```python
from build123d import *

# Parameters (mm, degrees)
BOSS_EXTRUDE1_DEPTH = 3.2
SKETCH8_R           = 2
CUT_EXTRUDE1_DEPTH  = 7.23083729


with BuildPart() as part:
    # Sketch1 → Boss-Extrude1 (new body)
    with BuildSketch(Plane(origin=(0, 0, 0), x_dir=(1, 0, 0), z_dir=(0, 1, 0))):
        Polygon((0, 4.041451884), (-3.5, 2.020725942), (-3.5, -2.020725942), (0, -4.041451884), (3.5, -2.020725942), (3.5, 2.020725942), align=None)
    extrude(amount=BOSS_EXTRUDE1_DEPTH)

    # Sketch3 → Cut-Revolve2 (revolve, cut)
    with BuildSketch(Plane(origin=(0, 0, 0), x_dir=(0.8660254037844417, 0, 0.4999999999999949), z_dir=(-0.4999999999999949, 0, 0.8660254037844417)), mode=Mode.PRIVATE) as cut_revolve2_sk:
        Polygon((4.041451884, 3.2), (4.041451884, 2.54), (3.381451884, 3.2), align=None)
        Polygon((4.041451884, 0), (4.041451884, 0.66), (3.381451884, 0), align=None)
    revolve(cut_revolve2_sk.sketch.rotate(Axis((0, -1.01584762, 0), (0, 1, 0)), 300), axis=Axis((0, -1.01584762, 0), (0, 1, 0)), mode=Mode.SUBTRACT)

    # Sketch8 → Cut-Extrude1 (cut, through all)
    with BuildSketch(Plane(origin=(0, 3.2, 0), x_dir=(1, 0, 0), z_dir=(0, 1, 0))):
        with Locations(Location((0, 0, 0), (0, 0, 270))):
            Circle(SKETCH8_R)
    extrude(amount=-CUT_EXTRUDE1_DEPTH, mode=Mode.SUBTRACT)


solid = part.part
```
The model under review builds one solid part; all positions refer to its coordinate system, in mm. Round coordinates to 2 decimals unless told otherwise and drop trailing zeros. Order: outer loops, then holes, each group sorted by start corner. A loop starts at its lowest first (then second) coordinate and runs counter-clockwise, first axis right, second up. Notation, with made-up numbers: (87.5, 51.5) -> (99.5, 51.5) arc R13 ccw to (99.5, 56.5) -> close; hole circle Ø5 at (70.25, 79). An arc over 180 degrees is marked (long way). One line per item, written item: value. Start each with the question number.
Q1. Clearance check with flat-ended pins moving along their axes: pin 1 Ø1 at (x, y) = (-0.5, 3) entering from +Z; pin 2 Ø1.5 at (x, y) = (-1, 1) entering from -Z. State where each tip first meets the part, or that it passes through.
Q2. Mouldability with a two-part tool opening along Z and no side actions: class faces 1 (the face through (1.726, 1.579, 3.045)), 2 (the face through (-1.726, 1.579, -3.045)), 3 (the face through (-2, 2, 0)) as released by +Z, released by -Z, zero draft, split by the parting line, or undercut.
Q3. Wall thickness on line 1 (X direction, y = 2.45, z = 0); line 2 (Z direction, x = -0.5, y = 0.65); line 3 (X direction, y = 0.55, z = 1.75): over which ranges is each line inside the solid? List them lowest first.
Q4. Take a section at B-B (y = 0.85). Write out the cut boundary in (x, z), and give its area (3 significant figures).
Q5. Take a section at A-A (z = 0). Write out the cut boundary in (x, y).
Reported:
1. pin 1: stops at z = 3.95
1. pin 2: stops at z = -3.9
2. face 1: released by +Z
2. face 2: released by -Z
2. face 3: undercut
3. line 1: x = -3.5 to -2, 2 to 3.5
3. line 2: z = -3.75 to -1.94, 1.94 to 3.75
3. line 3: x = -3.5 to -0.97, 0.97 to 3.5
4. outline: (-3.5, -2.02) -> (0, -4.04) -> (3.5, -2.02) -> (3.5, 2.02) -> (0, 4.04) -> (-3.5, 2.02) -> close; hole circle Ø4 at (0, 0)
4. area: 29.9 mm2
5. outline: (-3.5, 0.12) -> (-3.38, 0) -> (-2, 0) -> (-2, 3.2) -> (-3.38, 3.2) -> (-3.5, 3.08) -> close; (2, 0) -> (3.38, 0) -> (3.5, 0.12) -> (3.5, 3.08) -> (3.38, 3.2) -> (2, 3.2) -> close
